For this review, use the dimensioned drawing (mm, ordinates from the lowest corner) and the shaded views. A direction names the side the tool comes from. Give positions to 0.01 mm unless a question says otherwise; leave off trailing zeros. Loops run counter-clockwise (first coordinate to the right, second up) from the corner with the lowest first, then second, coordinate; pieces in that order, holes last. Notation, with made-up numbers: (59, 17.5) -> (64, 17.5) arc R15 cw to (64, 39.5) -> close; hole circle Ø5 at (-4, 56). An arc over 180 degrees is marked (long way). Write each question's results on one line, items separated by ' | '. Start each with the question number.
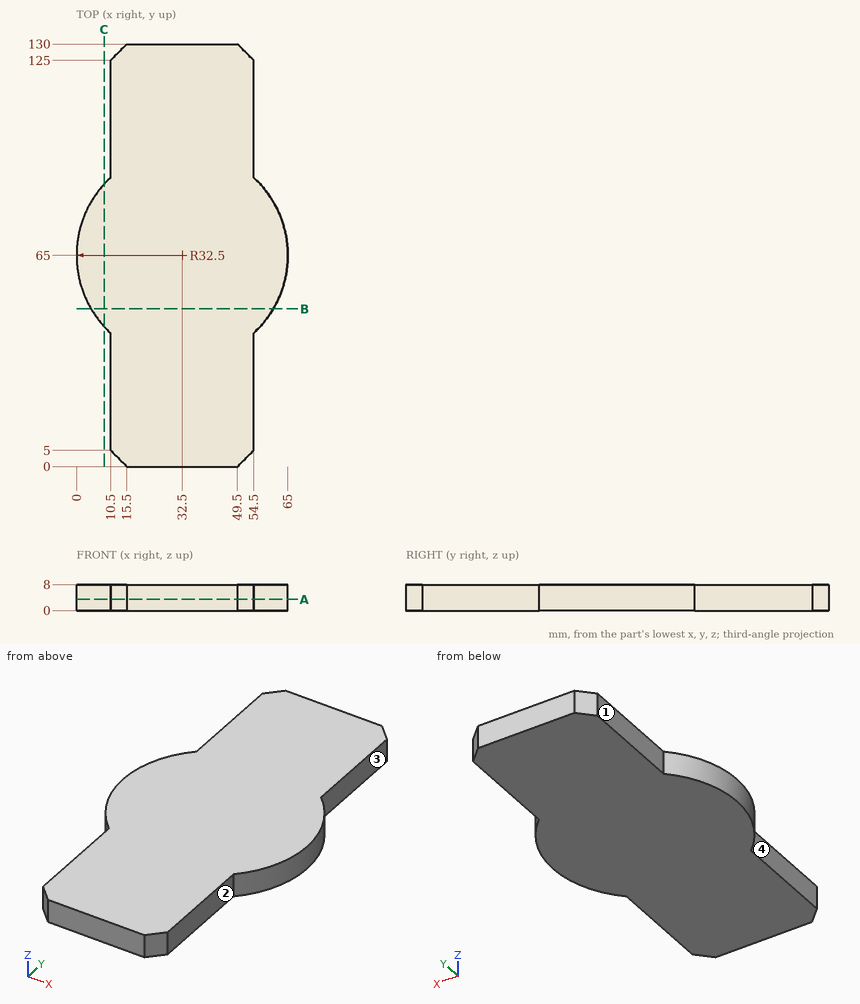
1. Machinability: for the marked faces 1, 2, 3 and 4, which of the approach directions +Z, -Z, +X, -X, +Y, -Y give a long, thin tool a straight path to every point of the face, cutting with its end or side? Answer none if there is none.
2. Wall thickness on L1, parallel to X at y = 116.5, z = 5; L2, parallel to X at y = 64.5, z = 5.75; L3, parallel to Y at x = 52, z = 7: over which ranges is each line inside the solid? List them lowest first.
3. We need section A-A (z = 3.5). Write out the cut boundary in (x, y), plus the area to 3 significant figures.
4. We need section C-C (x = 8.5). Write out the cut boundary in (y, z), plus the area to 3 significant figures.
5. We need section B-B (y = 48.5). Write out the cut boundary in (x, z).
Response:
1) face 1: +Z, -Z, -X, +Y | face 2: +Z, -Z, +X, -Y | face 3: +Z, -Z, +X, +Y | face 4: +Z, -Z, -X, -Y
2) L1: x = 10.5 to 54.5 | L2: x = 0 to 65 | L3: y = 2.5 to 127.5
3) outline: (10.5, 5) -> (15.5, 0) -> (49.5, 0) -> (54.5, 5) -> (54.5, 41.08) arc R32.5 ccw to (54.5, 88.92) -> (54.5, 125) -> (49.5, 130) -> (15.5, 130) -> (10.5, 125) -> (10.5, 88.92) arc R32.5 ccw to (10.5, 41.08) -> close | area: 6,360 mm2
4) outline: (43.09, 0) -> (86.91, 0) -> (86.91, 8) -> (43.09, 8) -> close | area: 351 mm2
5) outline: (4.5, 0) -> (60.5, 0) -> (60.5, 8) -> (4.5, 8) -> close
